from build123d import *

# Parameters (mm, degrees)
SKETCH1_W           = 84
SKETCH1_H           = 52
BOSS_EXTRUDE1_DEPTH = 20
SKETCH2_R           = 17.5
CUT_EXTRUDE1_DEPTH  = 20
SKETCH3_R           = 3
CUT_EXTRUDE2_DEPTH  = 20
SKETCH4_R           = 1.25
CUT_EXTRUDE3_DEPTH  = 20
SKETCH5_R           = 4
CUT_EXTRUDE4_DEPTH  = 20
SKETCH6_R           = 7
CUT_EXTRUDE5_DEPTH  = 7.8
CHAMFER1_SIZE       = 0.5


with BuildPart() as part:
    # Sketch1 → Boss-Extrude1 (new body)
    with BuildSketch(Plane(origin=(0, 0, 0), x_dir=(1, 0, 0), z_dir=(0, 1, 0))):
        Rectangle(SKETCH1_W, SKETCH1_H)
    extrude(amount=BOSS_EXTRUDE1_DEPTH)

    # Sketch2 → Cut-Extrude1 (cut)
    with BuildSketch(Plane(origin=(0, 20, 0), x_dir=(1, 0, 0), z_dir=(0, 1, 0))):
        with Locations(Location((-20, 0, 0), (0, 0, 270))):
            Circle(SKETCH2_R)
    extrude(amount=-CUT_EXTRUDE1_DEPTH, mode=Mode.SUBTRACT)

    # Sketch3 → Cut-Extrude2 (cut)
    with BuildSketch(Plane(origin=(0, 20, 0), x_dir=(1, 0, 0), z_dir=(0, 1, 0))):
        with Locations(Location((8, 8.5, 0), (0, 0, 270))):
            Circle(SKETCH3_R)
    extrude(amount=-CUT_EXTRUDE2_DEPTH, mode=Mode.SUBTRACT)

    # Sketch4 → Cut-Extrude3 (cut)
    with BuildSketch(Plane(origin=(0, 20, 0), x_dir=(1, 0, 0), z_dir=(0, 1, 0))):
        with Locations(Location((19.4, -18.6, 0), (0, 0, 270))):
            Circle(SKETCH4_R)
        with Locations(Location((38.6, 18.6, 0), (0, 0, 270))):
            Circle(SKETCH4_R)
    extrude(amount=-CUT_EXTRUDE3_DEPTH, mode=Mode.SUBTRACT)

    # Sketch5 → Cut-Extrude4 (cut)
    with BuildSketch(Plane(origin=(0, 20, 0), x_dir=(1, 0, 0), z_dir=(0, 1, 0))):
        with Locations(Location((29, 0, 0), (0, 0, 270))):
            Circle(SKETCH5_R)
    extrude(amount=-CUT_EXTRUDE4_DEPTH, mode=Mode.SUBTRACT)

    # Sketch6 → Cut-Extrude5 (cut)
    with BuildSketch(Plane(origin=(0, 20, 0), x_dir=(1, 0, 0), z_dir=(0, 1, 0))):
        with Locations(Location((29, 0, 0), (0, 0, 270))):
            Circle(SKETCH6_R)
    extrude(amount=-CUT_EXTRUDE5_DEPTH, mode=Mode.SUBTRACT)

    # Chamfer1
    chamfer1_edges = [part.edges().sort_by_distance(p)[0] for p in [
        (-42, 20, 0),
        (0, 20, 26),
        (42, 20, 0),
        (0, 0, 26),
        (-42, 0, 0),
        (0, 0, -26),
        (42, 0, 0),
        (0, 20, -26),
    ]]
    chamfer(chamfer1_edges, length=CHAMFER1_SIZE)


solid = part.part
Read the model definition and answer for the solid it produces. Units are mm, in the model's axes. A direction names the side the tool comes from. Give positions to 0.01 mm unless a question says otherwise; leave off trailing zeros. Write each loop counter-clockwise with the first axis right and the second up, starting at its lowest first coordinate (ties: lowest second). Pieces come first, ordered by that corner, then holes. Notation, with made-up numbers: (59, 60.5) -> (88, 60.5) arc R12 ccw to (88, 81.5) -> close; hole circle Ø5 at (70, -34.5). An arc over 180 degrees is marked (long way). Answer as a JSON object with one key per item and string values. Group by question number.
1) A tool of negligible diameter and unlimited length cuts with its end or side. For faces 1 (the flat face through (9, 0, 0)), 2 (the cylindrical face through (22.166, 16.155, -1.517)), from which of +Z, -Z, +X, -X, +Y, -Y can it reach the whole face along a straight path? Write none if from no direction.
2) Find section B-B (z = 18.6). Write down the section's boundary in (x, y), and give its area (3 significant figures).
3) Consider L1, parallel to X at y = 13.5, z = -18.6; L2, parallel to X at y = 8.75, z = 3; L3, parallel to X at y = 8.25, z = 18.6. Determine where each line is inside the solid, lowest interval first. Write a range as from..to.
4) Find section A-A (x = 8). Write down the section's boundary in (y, z).
5) Each of these flat-tipped pins is pushed along its axis until it touches: P1, Ø6.5, axis at x = 29, z = 0, coming from the +Y side; P2, Ø11, axis at x = 30, z = 0, coming from the +Y side. Where does it stop, or does it pass through?
6) Find section C-C (z = 0). Write down the section's boundary in (x, y), and give its area (3 significant figures).
7) The mould has two halves that part along Z. Classify faces 3 (the cylindrical face through (37.491, 10.14, -18.023)), 4 (the flat face through (-1, 10, 26)), 5 (the cylindrical face through (32.966, 6.185, -0.521)), 6 (the flat face through (-1, 20, 0)): +Z half, -Z half, draft (parallel to the pull), parting line (faces both ways), or undercut.
8) Find section D-D (y = 9.5). Write down the section's boundary in (x, z), and give its area (3 significant figures).
Values follow:
{
 "1": {"face 1": "+Z, -Z, +X, -X, -Y", "face 2": "+Y"},
 "2": {"outline": "(-42, 0.5) -> (-41.5, 0) -> (18.15, 0) -> (18.15, 20) -> (-41.5, 20) -> (-42, 19.5) -> close; (20.65, 0) -> (41.5, 0) -> (42, 0.5) -> (42, 19.5) -> (41.5, 20) -> (20.65, 20) -> close", "area": "1,630 mm2"},
 "3": {"L1": "x = -42..37.35, 39.85..42", "L2": "x = -42..-37.24, -2.76..26.35, 31.65..42", "L3": "x = -42..18.15, 20.65..42"},
 "4": {"outline": "(0, -25.5) -> (0.5, -26) -> (19.5, -26) -> (20, -25.5) -> (20, -11.5) -> (0, -11.5) -> close; (0, -5.5) -> (20, -5.5) -> (20, 25.5) -> (19.5, 26) -> (0.5, 26) -> (0, 25.5) -> close"},
 "5": {"P1": "passes through", "P2": "stops at y = 12.2"},
 "6": {"outline": "(-42, 0.5) -> (-41.5, 0) -> (-37.5, 0) -> (-37.5, 20) -> (-41.5, 20) -> (-42, 19.5) -> close; (-2.5, 0) -> (25, 0) -> (25, 12.2) -> (22, 12.2) -> (22, 20) -> (-2.5, 20) -> close; (33, 0) -> (41.5, 0) -> (42, 0.5) -> (42, 19.5) -> (41.5, 20) -> (36, 20) -> (36, 12.2) -> (33, 12.2) -> close", "area": "773 mm2"},
 "7": {"face 3": "undercut", "face 4": "+Z half", "face 5": "undercut", "face 6": "draft"},
 "8": {"outline": "(-42, -26) -> (42, -26) -> (42, 26) -> (-42, 26) -> close; hole circle Ø35 at (-20, 0); hole circle Ø6 at (8, -8.5); hole circle Ø2.5 at (19.4, 18.6); hole circle Ø8 at (29, 0); hole circle Ø2.5 at (38.6, -18.6)", "area": "3,320 mm2"}
}
